```python
from build123d import *

# Parameters (mm, degrees)
SKETCH1_R              = 44.5
BOSS_EXTRUDE1_DEPTH    = 1090
SKETCH2_R              = 10
BOSS_EXTRUDE2_DEPTH    = 13
BOSS_EXTRUDE3_START    = 13
SKETCH3_R              = 10
BOSS_EXTRUDE3_DEPTH    = 13
M12_TAPPED_HOLE1_D     = 10.2
M12_TAPPED_HOLE1_DEPTH = 25.25
M12_TAPPED_HOLE1_TIP   = 3.064389157
M12_TAPPED_HOLE2_D     = 10.2
M12_TAPPED_HOLE2_DEPTH = 25.25
M12_TAPPED_HOLE2_TIP   = 3.064389157


with BuildPart() as part:
    # Sketch1 → Boss-Extrude1 (new body)
    with BuildSketch(Plane.XY):
        Circle(SKETCH1_R)
    extrude(amount=BOSS_EXTRUDE1_DEPTH)

    # Sketch2 → Boss-Extrude2 (add)
    with BuildSketch(Plane.XY.offset(1090)):
        with Locations(Location((0, 0, 0), (0, 0, 180))):
            Circle(SKETCH2_R)
    extrude(amount=BOSS_EXTRUDE2_DEPTH)

    # Sketch3 → Boss-Extrude3 (add)
    with BuildSketch(Plane(origin=(0, 0, 0), x_dir=(-1, 0, 0), z_dir=(0, 0, -1)).offset(BOSS_EXTRUDE3_START)):
        Circle(SKETCH3_R)
    extrude(amount=-BOSS_EXTRUDE3_DEPTH)

    # M12 Tapped Hole1
    with Locations(Plane(origin=(0, 0, -13), x_dir=(-1, 0, 0), z_dir=(0, 0, -1))):
        with Locations((0, 0)):
            Hole(M12_TAPPED_HOLE1_D / 2, depth=M12_TAPPED_HOLE1_DEPTH)
            with Locations((0, 0, -(M12_TAPPED_HOLE1_DEPTH + M12_TAPPED_HOLE1_TIP / 2))):  # 118° drill point
                Cone(0, M12_TAPPED_HOLE1_D / 2, M12_TAPPED_HOLE1_TIP, mode=Mode.SUBTRACT)

    # M12 Tapped Hole2
    with Locations(Plane.XY.offset(1103)):
        with Locations((0, 0)):
            Hole(M12_TAPPED_HOLE2_D / 2, depth=M12_TAPPED_HOLE2_DEPTH)
            with Locations((0, 0, -(M12_TAPPED_HOLE2_DEPTH + M12_TAPPED_HOLE2_TIP / 2))):  # 118° drill point
                Cone(0, M12_TAPPED_HOLE2_D / 2, M12_TAPPED_HOLE2_TIP, mode=Mode.SUBTRACT)


solid = part.part
```
Verification items for the finished model (mm, model axes). A direction names the side the tool comes from. Round coordinates to 2 decimals unless told otherwise and drop trailing zeros. Order: outer loops, then holes, each group sorted by start corner. A loop starts at its lowest first (then second) coordinate and runs counter-clockwise, first axis right, second up.
1) Material ranges on line 1 (Y direction, x = 0, z = 5); line 2 (Y direction, x = 0, z = -3.5); line 3 (Z direction, x = -34, y = -24.5), recorded low to high.
Geometry says:
line 1: y = -44.5 to -5.1, 5.1 to 44.5
line 2: y = -10 to -5.1, 5.1 to 10
line 3: z = 0 to 1090
2) Tool access check on faces 1 (the flat face through (2, 5, -13)), 2 (the cylindrical face through (2.17, -9.76, -6.59)), 3 (the cylindrical face through (10, 0, 1096)). Record the directions out of +Z, -Z, +X, -X, +Y, -Y that give a thin tool (end or side, any length) a straight path to the whole face; none if there is none.
Geometry says:
face 1: -Z, +X, -X, +Y, -Y
face 2: -Z
face 3: +Z
3) Depth check by flat-ended pin: pin 1 (12 mm diameter, centred on y = -6.5, z = 950.5, fed in from +X); pin 2 (5 mm diameter, centred on x = -10.5, y = 27, fed in from -Z); pin 3 (8 mm diameter, centred on x = -34.5, z = 615.5, fed in from +Y). Enter the tip coordinate at first touch or a pass-through.
Geometry says:
pin 1: stops at x = 44.5
pin 2: stops at z = 0
pin 3: stops at y = 32.4
4) Cross-section at B-B, the plane y = -30.5. Record the cut outline in (x, z), plus the area to 3 significant figures.
Geometry says:
outline: (-32.4, 0) - (32.4, 0) - (32.4, 1090) - (-32.4, 1090) - close
area: 70,600 mm2
5) Cross-section at A-A, the plane z = 905. Record the cut outline in (x, y), plus the area to 3 significant figures.
Geometry says:
outline: circle Ø89 at (0, 0)
area: 6,220 mm2
6) Cross-section at C-C, the plane x = 20. Record the cut outline in (y, z).
Geometry says:
outline: (-39.75, 0) - (39.75, 0) - (39.75, 1090) - (-39.75, 1090) - close
